from build123d import *

# Parameters (mm, degrees)
SKETCH1_R          = 4
BOSS_EXTRU_1_DEPTH = 4


with BuildPart() as part:
    # Sketch1 → Boss.-Extru.1 (new body)
    with BuildSketch(Plane(origin=(0, 0, 0), x_dir=(1, 0, 0), z_dir=(0, 1, 0))):
        with BuildLine():
            Line((38.094109607, -47.888548123), (-43.540851016, 33.7464125))
            ThreePointArc((-43.540851016, 33.7464125), (-43.540851016, 47.888548123), (-29.398715392, 47.888548123))
            Line((-29.398715392, 47.888548123), (52.236245231, -33.7464125))
            ThreePointArc((52.236245231, -33.7464125), (52.236245231, -47.888548123), (38.094109607, -47.888548123))
        make_face()
        with Locations(Location((45.165177419, -40.817480312, 0), (0, 0, 270))):
            Circle(SKETCH1_R, mode=Mode.SUBTRACT)
        with Locations(Location((-36.469783204, 40.817480312, 0), (0, 0, 270))):
            Circle(SKETCH1_R, mode=Mode.SUBTRACT)
    extrude(amount=BOSS_EXTRU_1_DEPTH)


solid = part.part
Geometry check sheet. Reference: the model listing, model coordinates, mm. Give positions to 0.01 mm unless a question says otherwise; leave off trailing zeros. Order: outer loops, then holes, each group sorted by start corner. A loop starts at its lowest first (then second) coordinate and runs counter-clockwise, first axis right, second up.
1. Sectioned sample at C-C (x = 19). Record the boundary of the cut face in (y, z).
Completed:
outline: (0, 0.51) - (4, 0.51) - (4, 28.79) - (0, 28.79) - close
2. Scan lines: line 1 (X direction, y = 1.7, z = 44.5); line 2 (Z direction, x = -39, y = 2.5); line 3 (X direction, y = 1.75, z = 38). Record each from-to range of solid material in increasing order.
Completed:
line 1: x = 34.71 to 43.6, 46.73 to 54.46
line 2: z = -50.49 to -43.92, -37.72 to -29.21
line 3: x = 28.21 to 42.33, 48 to 54.76
3. Sectioned sample at B-B (z = -4.5). Record the boundary of the cut face in (x, y), then the cut area to 3 significant figures.
Completed:
outline: (-14.29, 0) - (13.99, 0) - (13.99, 4) - (-14.29, 4) - close
area: 113 mm2
4. Sectioned sample at A-A (y = 3.15). Record the boundary of the cut face in (x, z), then the cut area to 3 significant figures.
Completed:
outline: (-43.54, -33.75) arc R10 ccw to (-29.4, -47.89) - (52.24, 33.75) arc R10 ccw to (38.09, 47.89) - close; hole circle Ø8 at (-36.47, -40.82); hole circle Ø8 at (45.17, 40.82)
area: 2,520 mm2
5. Draft check along Z on faces 1 (the face through (5, 4, 0)), 2 (the face through (41.616, 1.972, 42.663)), 3 (the face through (52.39, 1.97, 47.73)), 4 (the face through (-38.904, 1.972, -43.992)). Enter one of: pulls with the +Z half, pulls with the -Z half, needs draft (parallel to the pull), parting line crosses it, or undercut.
Completed:
face 1: needs draft
face 2: undercut
face 3: parting line crosses it
face 4: undercut
6. Depth check by flat-ended pin: pin 1 (13 mm diameter, centred on x = -36.47, z = -40.82, fed in from -Y); pin 2 (2 mm diameter, centred on x = -24, y = 3.5, fed in from +Z); pin 3 (1 mm diameter, centred on x = -18.5, y = 2.5, fed in from -Z); pin 4 (1.5 mm diameter, centred on y = 3, z = 8.5, fed in from -X). Enter the tip coordinate at first touch or a pass-through.
Completed:
pin 1: stops at y = 0
pin 2: stops at z = -13.21
pin 3: stops at z = -37.49
pin 4: stops at x = -2.04
